Source: CAD feature listing. Evaluate the final solid. Frame: model axes, mm. Round coordinates to 2 decimals unless told otherwise and drop trailing zeros. Order: outer loops, then holes, each group sorted by start corner. A loop starts at its lowest first (then second) coordinate and runs counter-clockwise, first axis right, second up. Notation, with made-up numbers: (61.5, 23.25) - (83.5, 23.25) arc R25 cw to (83.5, 43.25) - close; hole circle Ø9 at (3.25, 21.25). An arc over 180 degrees is marked (long way). Return JSON: item names as keys, results as strings. Group by question number.
1) Contact query for flat-ended pins moving along their axis: P1, Ø9, axis at x = -8.79, y = -70.71, coming from the +Z side; P2, Ø5, axis at x = -200, y = -108, coming from the +Z side; P3, Ø2.5, axis at x = -82, y = -108.5, coming from the -Z side; P4, Ø2, axis at y = -59.5, z = 5.5, coming from the +X side. Output: stop coordinate, or through.
2) Section D-D, the plane x = -214. Return loops of the section in (y, z).
3) Section A-A, the plane x = 0. Return loops of the section in (y, z).
4) Ray query, line 1 (Y direction, x = -20, z = 0.95); line 2 (X direction, y = -40.5, z = 5); line 3 (X direction, y = -111.5, z = 2.5). Return the intervals inside material, ascending. Write a range as from..to.
5) Section B-B, the plane y = -17. Return loops of the section in (x, z).
6) Section C-C, the plane z = 10. Give the number of separate pieces and of enclosed holes in the cut face, plus the area to 4 significant figures.
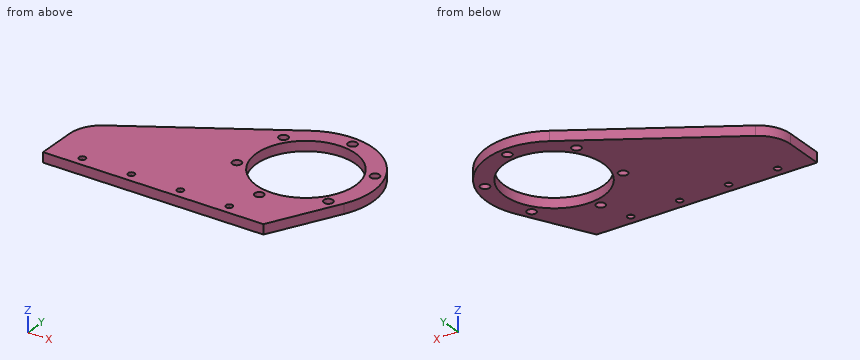
```python
from build123d import *

# Parameters (mm, degrees)
EXTRUDE_1_DEPTH     = 12
SKETCH_2_R          = 60.5
CUT_EXTRUDE_2_DEPTH = 269.596351427
SKETCH_3_R          = 2
CUT_EXTRUDE_3_DEPTH = 269.596351427
SKETCH_4_R          = 4
CUT_EXTRUDE_4_DEPTH = 4
CUT_EXTRUDE_START   = -4
SKETCH_5_R          = 4
CUT_EXTRUDE_5_DEPTH = 4
SKETCH_6_R          = 5.5
CUT_EXTRUDE_6_DEPTH = 269.596351427


with BuildPart() as part:
    # 草图1 → 凸台-拉伸1 (new body)
    with BuildSketch(Plane.XY):
        with BuildLine():
            Line((0, -120), (-240, -120))
            Line((-240, -120), (-240, -72.488505))
            ThreePointArc((-240, -72.488505), (-234.867302193, -52.885667507), (-220.786438112, -38.313602065))
            Line((-220.786438112, -38.313602065), (-42.612198129, 70.058551017))
            ThreePointArc((-42.612198129, 70.058551017), (56.016961424, 59.884054913), (72.743129476, -37.847550964))
            Line((72.743129476, -37.847550964), (30, -120))
            Line((30, -120), (0, -120))
        make_face()
    extrude(amount=EXTRUDE_1_DEPTH)

    # 草图2 → 切除-拉伸2 (cut, through all)
    with BuildSketch(Plane.XY):
        Circle(SKETCH_2_R)
    extrude(amount=CUT_EXTRUDE_2_DEPTH, mode=Mode.SUBTRACT)

    # 草图3 → 切除-拉伸3 (cut, through all)
    with BuildSketch(Plane.XY.offset(12)):
        with Locations((-200, -108)):
            Circle(SKETCH_3_R)
        with Locations((-140, -108)):
            Circle(SKETCH_3_R)
        with Locations((-80, -108)):
            Circle(SKETCH_3_R)
        with Locations((-20, -108)):
            Circle(SKETCH_3_R)
    extrude(amount=-CUT_EXTRUDE_3_DEPTH, mode=Mode.SUBTRACT)

    # 草图4 → 切除-拉伸4 (cut)
    with BuildSketch(Plane.XY.offset(12)):
        with Locations((-200, -108)):
            Circle(SKETCH_4_R)
        with Locations((-140, -108)):
            Circle(SKETCH_4_R)
        with Locations((-80, -108)):
            Circle(SKETCH_4_R)
        with Locations((-20, -108)):
            Circle(SKETCH_4_R)
    extrude(amount=-CUT_EXTRUDE_4_DEPTH, mode=Mode.SUBTRACT)

    # 草图5 → 切除-拉伸5 (cut)
    with BuildSketch(Plane(origin=(0, 0, 0), x_dir=(-1, 0, 0), z_dir=(0, 0, -1)).offset(CUT_EXTRUDE_START)):
        with Locations(Location((20, -108, 0), (0, 0, 180))):
            Circle(SKETCH_5_R)
        with Locations(Location((80, -108, 0), (0, 0, 180))):
            Circle(SKETCH_5_R)
        with Locations(Location((140, -108, 0), (0, 0, 180))):
            Circle(SKETCH_5_R)
        with Locations(Location((200, -108, 0), (0, 0, 180))):
            Circle(SKETCH_5_R)
    extrude(amount=CUT_EXTRUDE_5_DEPTH, mode=Mode.SUBTRACT)

    # 草图6 → 切除-拉伸6 (cut, through all)
    with BuildSketch(Plane(origin=(0, 0, 0), x_dir=(-1, 0, 0), z_dir=(0, 0, -1))):
        with Locations((56.836099532, 42.967665634)):
            Circle(SKETCH_6_R)
        with Locations((-8.793040215, 70.705338863)):
            Circle(SKETCH_6_R)
        with Locations((65.629139746, -27.737673229)):
            Circle(SKETCH_6_R)
        with Locations((8.793040215, -70.705338863)):
            Circle(SKETCH_6_R)
        with Locations((-56.836099532, -42.967665634)):
            Circle(SKETCH_6_R)
        with Locations((-65.629139746, 27.737673229)):
            Circle(SKETCH_6_R)
    extrude(amount=-CUT_EXTRUDE_6_DEPTH, mode=Mode.SUBTRACT)


solid = part.part
```
Geometry check:
{
 "1": {"P1": "through", "P2": "z = 8", "P3": "z = 4", "P4": "x = 62"},
 "2": {"outline": "(-120, 0) - (-34.19, 0) - (-34.19, 12) - (-120, 12) - close"},
 "3": {"outline": "(-120, 0) - (-60.5, 0) - (-60.5, 12) - (-120, 12) - close; (60.5, 0) - (82, 0) - (82, 12) - (60.5, 12) - close"},
 "4": {"line 1": "-120..-112, -104..-57.1, 57.1..79.52", "line 2": "-224.02..-44.94, 44.94..51.92, 61.75..71.36", "line 3": "-240..-201.94, -198.06..-141.94, -138.06..-81.94, -78.06..-21.94, -18.06..34.42"},
 "5": {"outline": "(-185.74, 0) - (-58.06, 0) - (-58.06, 12) - (-185.74, 12) - close; (58.06, 0) - (80.22, 0) - (80.22, 12) - (58.06, 12) - close"},
 "6": {"separate pieces": "1", "enclosed holes": "11", "area": "34,250 mm2"}
}
